Build history of the part. All positions in model axes, mm. Coordinates: 2 decimals unless noted, no trailing zeros. Order: outer loops, then holes, each group sorted by start corner. A loop starts at its lowest first (then second) coordinate and runs counter-clockwise, first axis right, second up. Notation, with made-up numbers: (39.5, 5.25) - (62.5, 5.25) arc R33 ccw to (62.5, 37.25) - close; hole circle Ø9 at (47.25, -1.5). An arc over 180 degrees is marked (long way). Write each question's results on one line, items separated by ' | '. Start each with the question number.
from build123d import *

# Parameters (mm, degrees)
SKETCH_1_R          = 60
SKETCH_1_R_2        = 25
EXTRUDE_1_DEPTH     = 20
CHAMFER_1_SIZE      = 10
SKETCH_2_R          = 1.5
CUT_EXTRUDE_1_DEPTH = 27


with BuildPart() as part:
    # 草图1 → 凸台-拉伸1 (new body)
    with BuildSketch(Plane.XY):
        Circle(SKETCH_1_R)
        Circle(SKETCH_1_R_2, mode=Mode.SUBTRACT)
    extrude(amount=EXTRUDE_1_DEPTH)

    # 倒角1
    chamfer_1_edges = [part.edges().sort_by_distance(p)[0] for p in [
        (-25, 0, 0),
    ]]
    chamfer(chamfer_1_edges, length=CHAMFER_1_SIZE)

    # 草图2 → 切除-拉伸1 (cut)
    with BuildSketch(Plane.XY.offset(20)):
        with Locations((0, 55)):
            Circle(SKETCH_2_R)
        with Locations((55, 0)):
            Circle(SKETCH_2_R)
        with Locations((0, -55)):
            Circle(SKETCH_2_R)
        with Locations((-55, 0)):
            Circle(SKETCH_2_R)
    extrude(amount=-CUT_EXTRUDE_1_DEPTH, mode=Mode.SUBTRACT)


solid = part.part
Item 1: Pull direction Y, two halves, no side cores. Call faces 1 (the flat face through (-1, -26, 20)), 2 (the cylindrical face through (-1.2, 54.1, 10.1)), 3 (the cylindrical face through (-59.94, 2.64, 9.86)): released by +Y, released by -Y, zero draft, split by the parting line, or undercut.
Item 2: Slice it at C-C (y = 55). Write the cut outline in (x, z).
Item 3: Probe probe 1 along Y at (x, z) = (0, 17.5); probe 2 along X at (y, z) = (-25, 3.25); probe 3 along Y at (x, z) = (12, 10.25). List the from-to ranges inside material, lowest first.
Item 4: Flat gauge pins, fed straight in: P1, Ø8, axis at x = -23.5, z = 7, coming from the -Y side; P2, Ø10, axis at y = -35, z = 11, coming from the -X side; P3, Ø2, axis at x = 2, z = 14.5, coming from the +Y side. Where does each tip first touch, or does it go through?
Item 5: Slice it at A-A (x = 0). Write the cut outline in (y, z), then the cut area to 3 significant figures.
Item 6: Slice it at B-B (z = 15). Write the cut outline in (x, y), then the cut area to 3 significant figures.
Resolved:
1) face 1: zero draft | face 2: undercut | face 3: split by the parting line
2) outline: (-23.98, 0) - (-1.5, 0) - (-1.5, 20) - (-23.98, 20) - close; (1.5, 0) - (23.98, 0) - (23.98, 20) - (1.5, 20) - close
3) probe 1: -60 to -56.5, -53.5 to -25, 25 to 53.5, 56.5 to 60 | probe 2: -54.54 to -19.57, 19.57 to 54.54 | probe 3: -58.79 to -21.93, 21.93 to 58.79
4) P1: y = -56.74 | P2: x = -51.96 | P3: y = 59.99
5) outline: (-60, 0) - (-56.5, 0) - (-56.5, 20) - (-60, 20) - close; (-53.5, 0) - (-35, 0) - (-25, 10) - (-25, 20) - (-53.5, 20) - close; (25, 10) - (35, 0) - (53.5, 0) - (53.5, 20) - (25, 20) - close; (56.5, 0) - (60, 0) - (60, 20) - (56.5, 20) - close | area: 1,180 mm^2
6) outline: circle Ø120 at (0, 0); hole circle Ø3 at (-55, 0); hole circle Ø50 at (0, 0); hole circle Ø3 at (0, -55); hole circle Ø3 at (0, 55); hole circle Ø3 at (55, 0) | area: 9,320 mm^2
